```python
from build123d import *

# Parameters (mm, degrees)
SIDE_RECESS_SKETCH_33_R   = 16.5
SIDE_RECESS_SKETCH_33_R_2 = 5
SIDE_RECESS_33X5_DEPTH    = 5


with BuildPart() as part:
    # Wheel Profile Sketch → Wheel Body (revolve)
    with BuildSketch(Plane.XY, mode=Mode.PRIVATE) as wheel_body_sk:
        Polygon((-7.5, -3.125), (7.5, -3.125), (7.5, -20), (3.5, -20), (0, -16.514784956), (-3.5, -20), (-7.5, -20), align=None)
    revolve(wheel_body_sk.sketch.rotate(Axis((0, 0, 0), (1, 0, 0)), 270), axis=Axis((0, 0, 0), (1, 0, 0)))

    # Side Recess Sketch Ø33 → Side Recess Ø33x5 (cut)
    with BuildSketch(Plane(origin=(7.5, 0, 0), x_dir=(0, 0, -1), z_dir=(1, 0, 0))):
        Circle(SIDE_RECESS_SKETCH_33_R)
        Circle(SIDE_RECESS_SKETCH_33_R_2, mode=Mode.SUBTRACT)
    side_recess_33x5 = extrude(amount=-SIDE_RECESS_33X5_DEPTH, mode=Mode.SUBTRACT)

    # Side Recess Mirror: Side Recess Ø33x5 across plane
    add(side_recess_33x5.mirror(Plane(origin=(0, 0, 0), x_dir=(0, 0, 1), z_dir=(1, 0, 0))), mode=Mode.SUBTRACT)


solid = part.part
```
Input: part model. Units: mm. Frame: model coordinates. A direction names the side the tool comes from. Coordinates: 2 decimals unless noted, no trailing zeros. Write each loop counter-clockwise with the first axis right and the second up, starting at its lowest first coordinate (ties: lowest second). Pieces come first, ordered by that corner, then holes. Notation, with made-up numbers: (54, 87) -> (93, 87) arc R17 ccw to (93, 119) -> close; hole circle Ø2 at (87, 15.25). An arc over 180 degrees is marked (long way). Write each question's results on one line, items separated by ' | '.
Item 1: Material intervals for probe 1 along Y at (x, z) = (-5.5, 0) (3 decimals); probe 2 along Y at (x, z) = (-6.5, -4); probe 3 along X at (y, z) = (7, 9), sorted ascending.
Conclusion:
probe 1: y = -20 to -16.5, -5 to -3.125, 3.125 to 5, 16.5 to 20 | probe 2: y = -19.6 to -16.01, -3 to 3, 16.01 to 19.6 | probe 3: x = -2.5 to 2.5
Item 2: Pin query (flat end, axial travel): pin 1 Ø1.5 at (y, z) = (2, 0.5) entering from +X; pin 2 Ø1 at (x, z) = (-1, -7.5) entering from +Y; pin 3 Ø8 at (x, z) = (-4, -4) entering from +Y; pin 4 Ø4 at (x, z) = (-2.5, -10) entering from -Y. Return the tip coordinate at first contact, or that it passes through.
Conclusion:
pin 1: passes through | pin 2: stops at y = 16.42 | pin 3: stops at y = 20 | pin 4: stops at y = -18.21
Item 3: Mould query, pull axis X, two halves, no side actions, for faces 1 (the conical face through (0.17, 16.287, -3.617)), 2 (the cylindrical face through (-5.528, 19.524, -4.336)), 3 (the flat face through (-7.5, -16.4, 2.9)). Classes: +X half, -X half, draft (parallel to the pull), parting line (faces both ways), or undercut.
Conclusion:
face 1: undercut | face 2: draft | face 3: -X half
Item 4: Section query C-C on x = -3. Return loops of the section in (y, z) (3 decimals), plus the area to 3 significant figures.
Conclusion:
outline: circle Ø39.004 at (0, 0); circle Ø10 at (0, 0); hole circle Ø33 at (0, 0); hole circle Ø6.25 at (0, 0) | area: 387 mm^2
Item 5: Section query D-D on x = 0.5. Return loops of the section in (y, z) (3 decimals), plus the area to 3 significant figures.
Conclusion:
outline: circle Ø34.025 at (0, 0); hole circle Ø6.25 at (0, 0) | area: 879 mm^2
Item 6: Set-up query: faces 4 (the cylindrical face through (5.472, 19.524, -4.336)), 5 (the cylindrical face through (-5.04, -6.32, -15.24)), 6 (the flat face through (7.5, 3.3, 0.1)), 7 (the conical face through (-0.219, 16.335, -3.627)), 8 (the cylindrical face through (5.04, -6.32, -15.24)). Return all of +Z, -Z, +X, -X, +Y, -Y with unobstructed straight access to the full face (end or side cutting, diameter ignored); none if empty.
Conclusion:
face 4: +X, -X | face 5: -X | face 6: +Z, -Z, +X, +Y, -Y | face 7: none | face 8: +X
